Work out the finished part from the listing and answer in its coordinate system (mm). A direction names the side the tool comes from. Round coordinates to 2 decimals unless told otherwise and drop trailing zeros. Write each loop counter-clockwise with the first axis right and the second up, starting at its lowest first coordinate (ties: lowest second). Pieces come first, ordered by that corner, then holes. Notation, with made-up numbers: M 72.25,78.25 L 131.25,78.25 A20 ccw 131.25,82.25 Z; hole C 84,-3 d9. An arc over 180 degrees is marked long. Answer in a Markdown table with one row per item.
```python
from build123d import *

# Parameters (mm, degrees)
BOSS_EXTRUDE1_DEPTH          = 478
CUT_EXTRUDE1_DEPTH           = 478
M12_TAPPED_HOLE1_D           = 10.2
M12_TAPPED_HOLE1_CSINK_D     = 12.05
M12_TAPPED_HOLE1_CSINK_ANGLE = 90
CUT_EXTRUDE2_DEPTH           = 478
M12_TAPPED_HOLE2_D           = 10.2
M12_TAPPED_HOLE2_CSINK_D     = 12.05
M12_TAPPED_HOLE2_CSINK_ANGLE = 90


with BuildPart() as part:
    # Sketch1 → Boss-Extrude1 (new body)
    with BuildSketch(Plane(origin=(0, 0, 0), x_dir=(1, 0, 0), z_dir=(0, 1, 0))):
        with BuildLine():
            Line((2489.747313266, 1503.388237), (2505.747313266, 1503.388237))
            Line((2505.747313266, 1503.388237), (2505.747313266, 1707.687544505))
            ThreePointArc((2505.747313266, 1707.687544505), (2499.07328063, 1727.247589931), (2481.835102198, 1738.648611511))
            Line((2481.835102198, 1738.648611511), (2268.738706702, 1794.314608702))
            Line((2268.738706702, 1794.314608702), (2264.694812236, 1778.834075199))
            Line((2264.694812236, 1778.834075199), (2465.835102198, 1726.291305576))
            ThreePointArc((2465.835102198, 1726.291305576), (2483.07328063, 1714.890283996), (2489.747313266, 1695.33023857))
            Line((2489.747313266, 1695.33023857), (2489.747313266, 1503.388237))
        make_face()
    extrude(amount=BOSS_EXTRUDE1_DEPTH)

    # Sketch2 → Cut-Extrude1 (cut)
    with BuildSketch(Plane(origin=(2505.747313266, 0, 0), x_dir=(0, 0, -1), z_dir=(1, 0, 0))):
        with BuildLine():
            Line((1563.688237, 81.6), (1603.288237, 81.6))
            ThreePointArc((1603.288237, 81.6), (1624.71357247, 90.47466453), (1633.588237, 111.9))
            Line((1633.588237, 111.9), (1633.588237, 366.1))
            ThreePointArc((1633.588237, 366.1), (1624.71357247, 387.52533547), (1603.288237, 396.4))
            Line((1603.288237, 396.4), (1563.688237, 396.4))
            ThreePointArc((1563.688237, 396.4), (1542.26290153, 387.52533547), (1533.388237, 366.1))
            Line((1533.388237, 366.1), (1533.388237, 111.9))
            ThreePointArc((1533.388237, 111.9), (1542.26290153, 90.47466453), (1563.688237, 81.6))
        make_face()
    extrude(amount=-CUT_EXTRUDE1_DEPTH, mode=Mode.SUBTRACT)

    # M12 Tapped Hole1 (through all)
    with Locations(Plane(origin=(2505.747313266, 0, 0), x_dir=(0, 0, -1), z_dir=(1, 0, 0))):
        with Locations((1633.588237, 416.55), (1533.388237, 61.45), (1533.388237, 416.55), (1633.588237, 61.45)):
            CounterSinkHole(M12_TAPPED_HOLE1_D / 2, M12_TAPPED_HOLE1_CSINK_D / 2, counter_sink_angle=M12_TAPPED_HOLE1_CSINK_ANGLE)

    # Sketch7 → Cut-Extrude2 (cut)
    with BuildSketch(Plane(origin=(583.702793267, 0, -2234.487255477), x_dir=(-0.9675333439556839, 0, -0.2527434041353648), z_dir=(0.2527434041353648, 0, -0.967533343955684))):
        with BuildLine():
            Line((-1741.579165164, 463), (-1741.579165164, 15))
            Line((-1741.579165164, 15), (-1853.078764419, 46.9719956))
            ThreePointArc((-1853.078764419, 46.9719956), (-1910.190162861, 86.223572269), (-1932.179165164, 151.941772797))
            Line((-1932.179165164, 151.941772797), (-1932.179165164, 326.058227203))
            ThreePointArc((-1932.179165164, 326.058227203), (-1910.190162861, 391.776427731), (-1853.078764419, 431.0280044))
            Line((-1853.078764419, 431.0280044), (-1741.579165164, 463))
        make_face()
    extrude(amount=-CUT_EXTRUDE2_DEPTH, mode=Mode.SUBTRACT)

    # M12 Tapped Hole2 (through all)
    with Locations(Plane(origin=(583.702793267, 0, -2234.487255477), x_dir=(-0.9675333439556839, 0, -0.2527434041353648), z_dir=(0.2527434041353648, 0, -0.967533343955684))):
        with Locations((-1901.479165164, 450), (-1901.479165164, 28)):
            CounterSinkHole(M12_TAPPED_HOLE2_D / 2, M12_TAPPED_HOLE2_CSINK_D / 2, counter_sink_angle=M12_TAPPED_HOLE2_CSINK_ANGLE)


solid = part.part
```
1. The part is cut by section A-A (z = -1585.5). Determine the outline of the cut face in (x, y), plus the area to 3 significant figures.
Calculated:
| item | result |
|---|---|
| outline | M 2489.75,0 L 2505.75,0 L 2505.75,81.6 L 2489.75,81.6 Z; M 2489.75,396.4 L 2505.75,396.4 L 2505.75,478 L 2489.75,478 Z |
| area | 2,610 mm² |
2. Consider line 1 along Z through (x, y) = (2493.5, 416.55); line 2 along Z through (x, y) = (2498, 61.45); line 3 along X through (y, z) = (162, -1523). Determine where each line is inside the solid, lowest interval first. Write a range as from..to.
Calculated:
| item | result |
|---|---|
| line 1 | z = -1732.86..-1638.69, -1628.49..-1538.49, -1528.29..-1503.39 |
| line 2 | z = -1728.56..-1638.69, -1628.49..-1538.49, -1528.29..-1503.39 |
| line 3 | x = 2489.75..2505.75 |
3. The part is cut by section D-D (y = 416.55). Determine the outline of the cut face in (x, z), plus the area to 3 significant figures.
Calculated:
| item | result |
|---|---|
| outline | M 2402.59,-1742.81 L 2406.63,-1758.29 L 2481.84,-1738.65 A32 ccw 2505.75,-1707.69 L 2505.75,-1639.61 L 2504.82,-1638.69 L 2489.75,-1638.69 L 2489.75,-1695.33 A32 cw 2465.84,-1726.29 Z; M 2489.75,-1628.49 L 2504.82,-1628.49 L 2505.75,-1627.56 L 2505.75,-1539.41 L 2504.82,-1538.49 L 2489.75,-1538.49 Z; M 2489.75,-1528.29 L 2504.82,-1528.29 L 2505.75,-1527.36 L 2505.75,-1503.39 L 2489.75,-1503.39 Z |
| area | 4,780 mm² |
4. Determine the mould class of faces 1 (the cylindrical face through (2482.892, 235.654, -1715.123)), 2 (the flat face through (2321.4, 446.8, -1772.4)), 3 (the flat face through (2498, 237, -1633.588)) for opening direction Z: released by +Z, released by -Z, zero draft, split by the parting line, or undercut.
Calculated:
| item | result |
|---|---|
| face 1 | released by +Z |
| face 2 | released by -Z |
| face 3 | undercut |
5. The part is cut by section C-C (y = 97). Determine the outline of the cut face in (x, z).
Calculated:
| item | result |
|---|---|
| outline | M 2434.76,-1734.41 L 2438.8,-1749.89 L 2481.84,-1738.65 A32 ccw 2505.75,-1707.69 L 2505.75,-1629.67 L 2489.75,-1629.67 L 2489.75,-1695.33 A32 cw 2465.84,-1726.29 Z; M 2489.75,-1537.3 L 2505.75,-1537.3 L 2505.75,-1503.39 L 2489.75,-1503.39 Z |
6. A tool of negligible diameter and unlimited length cuts with its end or side. For faces 4 (the flat face through (2489.747, 236, -1643)), 5 (the cylindrical face through (2497.859, 90.24, -1624.477)), 6 (the cylindrical face through (2425.99, 451.53, -1744.38)), from which of +Z, -Z, +X, -X, +Y, -Y can it reach the whole face along a straight path? Write none if from no direction.
Calculated:
| item | result |
|---|---|
| face 4 | +Z, -X, +Y, -Y |
| face 5 | +X, -X |
| face 6 | none |
7. The part is cut by section B-B (x = 2284). Determine the outline of the cut face in (y, z), plus the area to 3 significant figures.
Calculated:
| item | result |
|---|---|
| outline | M 0,-1790.33 L 19.52,-1790.33 L 20.72,-1773.79 L 0,-1773.79 Z; M 457.28,-1773.79 L 458.48,-1790.33 L 478,-1790.33 L 478,-1773.79 Z |
| area | 666 mm² |
8. Given pin 1 (2 mm diameter, centred on y = 289.5, z = -1667.5, fed in from -X); pin 2 (6 mm diameter, centred on y = 61.45, z = -1533.39, fed in from -X); pin 3 (17.5 mm diameter, centred on x = 2501.5, z = -1591.5, fed in from -Y); pin 4 (8 mm diameter, centred on x = 2496.5, y = 266.5, fed in from -Z), each flat-ended and moving along its own axis, determine where each tip first touches the part or whether it passes through.
Calculated:
| item | result |
|---|---|
| pin 1 | stops at x = 2489.75 |
| pin 2 | passes through |
| pin 3 | stops at y = 0 |
| pin 4 | stops at z = -1733.62 |
